CAD build for the part. Positions are in the model's coordinates, mm. Face numbers are marked on the shaded views. A direction names the side the tool comes from. Coordinates: 2 decimals unless noted, no trailing zeros. Write each loop counter-clockwise with the first axis right and the second up, starting at its lowest first coordinate (ties: lowest second). Pieces come first, ordered by that corner, then holes. Notation, with made-up numbers: (-2.75, 31.25) - (48.25, 31.25) arc R8 cw to (48.25, 37.25) - close; hole circle Ø9 at (73, 50.25). An arc over 180 degrees is marked (long way). One line per question, with ' | ' between items. Start each with the question number.
1. Flat gauge pins, fed straight in: P1, Ø5.5, axis at y = 33.25, z = 0, coming from the -X side; P2, Ø4, axis at y = 34, z = 1, coming from the +X side; P3, Ø1, axis at y = 16.5, z = -2, coming from the +X side. Where does each tip first touch, or does it go through?
2. Which spindle directions (+Z, -Z, +X, -X, +Y, -Y) get a long thin tool onto all of the face, cutting with end or side? Do the marked faces 4, 5 and 6. Say none if no direction does.
3. Band-saw the part on C-C, the plane y = 33.25. Write the cut outline in (x, z).
4. Band-saw the part on B-B, the plane x = -16. Write the cut outline in (y, z), then the cut area to 3 significant figures.
5. Two-plate mould, pull along X, no slides. Class the marked faces 1, 2 and 3: +X half, -X half, draft (parallel to the pull), parting line (faces both ways), or undercut.
6. Band-saw the part on A-A, the plane y = 23. Write the cut outline in (x, z).
7. Band-saw the part on D-D, the plane z = 4.75. Write the cut outline in (x, y).
8. Probe line 1 (Y direction, x = -7.5, z = 0); line 2 (X direction, y = 36.5, z = -4.5); line 3 (Z direction, x = -16, y = 4). List the from-to ranges inside material, lowest first.
from build123d import *

# Parameters (mm, degrees)
EXTRUDE_1_DEPTH           = 7
HOLE_WIZARD_1_D           = 4.4
HOLE_WIZARD_1_DEPTH       = 9.5
HOLE_WIZARD_1_CBORE_D     = 8
HOLE_WIZARD_1_CBORE_DEPTH = 4.4
HOLE_WIZARD_1_2_D         = 5.5
HOLE_WIZARD_1_3_D         = 3.2


with BuildPart() as part:
    # 草图1 → 凸台-拉伸1 (new, symmetric)
    with BuildSketch(Plane.XY):
        with BuildLine():
            Line((21, 0), (-21, 0))
            Line((-21, 0), (-21, 6))
            Line((-21, 6), (-10, 6))
            Line((-10, 6), (-10, 37.5))
            Line((-10, 37.5), (-0.5, 37.5))
            Line((-0.5, 37.5), (-0.5, 28.979130372))
            ThreePointArc((-0.5, 28.979130372), (0, 17), (0.5, 28.979130372))
            Line((0.5, 28.979130372), (0.5, 37.5))
            Line((0.5, 37.5), (10, 37.5))
            Line((10, 37.5), (10, 6))
            Line((10, 6), (21, 6))
            Line((21, 6), (21, 0))
        make_face()
    extrude(amount=EXTRUDE_1_DEPTH, both=True)

    # Hole Wizard 1
    with Locations(Plane(origin=(10, 0, 0), x_dir=(0, 0, -1), z_dir=(1, 0, 0))):
        with Locations((0, 33.25)):
            CounterBoreHole(HOLE_WIZARD_1_D / 2, HOLE_WIZARD_1_CBORE_D / 2, HOLE_WIZARD_1_CBORE_DEPTH, depth=HOLE_WIZARD_1_DEPTH)

    # Hole Wizard 1 2 (through all)
    with Locations(Plane(origin=(0, 6, 0), x_dir=(1, 0, 0), z_dir=(0, 1, 0))):
        with Locations((-16, 0), (16, 0)):
            Hole(HOLE_WIZARD_1_2_D / 2)

    # Hole Wizard 1 3 (through all)
    with Locations(Plane(origin=(-0.5, 0, 0), x_dir=(0, 0, -1), z_dir=(1, 0, 0))):
        with Locations((0, 33.25)):
            Hole(HOLE_WIZARD_1_3_D / 2)


solid = part.part
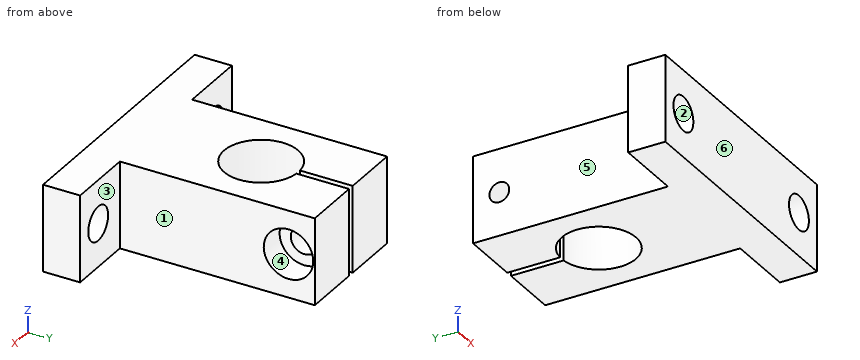
Filled in:
1) P1: stops at x = -10 | P2: stops at x = 5.6 | P3: stops at x = 10
2) face 4: +X | face 5: +Z, -Z, -X, +Y | face 6: +Z, -Z, +X, -X, -Y
3) outline: (-10, -7) - (-0.5, -7) - (-0.5, -1.6) - (-10, -1.6) - close; (-10, 1.6) - (-0.5, 1.6) - (-0.5, 7) - (-10, 7) - close; (0.5, -7) - (10, -7) - (10, -4) - (5.6, -4) - (5.6, -2.2) - (0.5, -2.2) - close; (0.5, 2.2) - (5.6, 2.2) - (5.6, 4) - (10, 4) - (10, 7) - (0.5, 7) - close
4) outline: (0, -7) - (6, -7) - (6, -2.75) - (0, -2.75) - close; (0, 2.75) - (6, 2.75) - (6, 7) - (0, 7) - close | area: 51.0 mm²
5) face 1: +X half | face 2: undercut | face 3: draft
6) outline: (-10, -7) - (-6, -7) - (-6, 7) - (-10, 7) - close; (6, -7) - (10, -7) - (10, 7) - (6, 7) - close
7) outline: (-21, 0) - (21, 0) - (21, 6) - (10, 6) - (10, 37.5) - (0.5, 37.5) - (0.5, 28.98) arc R6 cw (long way) to (-0.5, 28.98) - (-0.5, 37.5) - (-10, 37.5) - (-10, 6) - (-21, 6) - close
8) line 1: y = 0 to 31.65, 34.85 to 37.5 | line 2: x = -10 to -0.5, 0.5 to 10 | line 3: z = -7 to -2.75, 2.75 to 7
